from build123d import *

# Parameters (mm, degrees)
PLATE_OUTLINE_SKETCH_R = 10
BASE_PLATE_DEPTH       = 30
POCKET_SKETCH_R        = 10
POCKET_DEPTH           = 5


with BuildPart() as part:
    # Plate Outline Sketch → Base Plate (new body)
    with BuildSketch(Plane(origin=(0, 0, 0), x_dir=(1, 0, 0), z_dir=(0, 1, 0))):
        with BuildLine():
            ThreePointArc((-90, -88), (-80.846522891, -104.803361008), (-61.764705882, -106.225803982))
            ThreePointArc((-61.764705882, -106.225803982), (0, -92.919333848), (61.764705882, -106.225803982))
            ThreePointArc((61.764705882, -106.225803982), (80.846522891, -104.803361008), (90, -88))
            Line((90, -88), (90, -31.013960492))
            ThreePointArc((90, -31.013960492), (86.763523469, -20.105968885), (78.101571911, -12.728323162))
            Line((78.101571911, -12.728323162), (8.101571911, 18.28563733))
            ThreePointArc((8.101571911, 18.28563733), (0, 20), (-8.101571911, 18.28563733))
            Line((-8.101571911, 18.28563733), (-78.101571911, -12.728323162))
            ThreePointArc((-78.101571911, -12.728323162), (-86.763523469, -20.105968885), (-90, -31.013960492))
            Line((-90, -31.013960492), (-90, -88))
        make_face()
        with Locations(Location((70, -88, 0), (0, 0, 270))):
            Circle(PLATE_OUTLINE_SKETCH_R, mode=Mode.SUBTRACT)
        with Locations(Location((-70, -88, 0), (0, 0, 270))):
            Circle(PLATE_OUTLINE_SKETCH_R, mode=Mode.SUBTRACT)
        with Locations(Location((0, 0, 0), (0, 0, 270))):
            Circle(PLATE_OUTLINE_SKETCH_R, mode=Mode.SUBTRACT)
        with BuildLine():
            ThreePointArc((55.144271878, -90.075413685), (61.617206501, -75.560997904), (77.5, -75.009618943))
            ThreePointArc((77.5, -75.009618943), (82.5, -75.009618943), (85, -70.679491924))
            Line((85, -70.679491924), (85, -35.770992672))
            ThreePointArc((85, -35.770992672), (81.864151045, -25.019229582), (73.439959048, -17.639056998))
            Line((73.439959048, -17.639056998), (22.032686199, 6.289732813))
            ThreePointArc((22.032686199, 6.289732813), (17.05201209, 5.850545589), (14.942022328, 1.317561671))
            ThreePointArc((14.942022328, 1.317561671), (0, -15), (-14.942022328, 1.317561671))
            ThreePointArc((-14.942022328, 1.317561671), (-17.05201209, 5.850545589), (-22.032686199, 6.289732813))
            Line((-22.032686199, 6.289732813), (-73.439959048, -17.639056998))
            ThreePointArc((-73.439959048, -17.639056998), (-81.864151045, -25.019229582), (-85, -35.770992672))
            Line((-85, -35.770992672), (-85, -70.679491924))
            ThreePointArc((-85, -70.679491924), (-82.5, -75.009618943), (-77.5, -75.009618943))
            ThreePointArc((-77.5, -75.009618943), (-61.617206501, -75.560997904), (-55.144271878, -90.075413685))
            ThreePointArc((-55.144271878, -90.075413685), (-53.374733144, -94.623708504), (-48.573254036, -95.497808883))
            ThreePointArc((-48.573254036, -95.497808883), (0, -87.415527975), (48.573254036, -95.497808883))
            ThreePointArc((48.573254036, -95.497808883), (53.374733144, -94.623708504), (55.144271878, -90.075413685))
        make_face(mode=Mode.SUBTRACT)
    extrude(amount=BASE_PLATE_DEPTH)

    # Pocket Sketch → Pocket (add)
    with BuildSketch(Plane.XZ):
        with BuildLine():
            Line((-90, 88), (-90, 31.013960492))
            ThreePointArc((-90, 31.013960492), (-86.763523469, 20.105968885), (-78.101571911, 12.728323162))
            Line((-78.101571911, 12.728323162), (-8.101571911, -18.28563733))
            ThreePointArc((-8.101571911, -18.28563733), (0, -20), (8.101571911, -18.28563733))
            Line((8.101571911, -18.28563733), (78.101571911, 12.728323162))
            ThreePointArc((78.101571911, 12.728323162), (86.763523469, 20.105968885), (90, 31.013960492))
            Line((90, 31.013960492), (90, 88))
            ThreePointArc((90, 88), (80.846522891, 104.803361008), (61.764705882, 106.225803982))
            ThreePointArc((61.764705882, 106.225803982), (0, 92.919333848), (-61.764705882, 106.225803982))
            ThreePointArc((-61.764705882, 106.225803982), (-80.846522891, 104.803361008), (-90, 88))
        make_face()
        with Locations(Location((-70, 88, 0), (0, 0, 90))):
            Circle(POCKET_SKETCH_R, mode=Mode.SUBTRACT)
        with Locations(Location((0, 0, 0), (0, 0, 90))):
            Circle(POCKET_SKETCH_R, mode=Mode.SUBTRACT)
        with Locations(Location((70, 88, 0), (0, 0, 90))):
            Circle(POCKET_SKETCH_R, mode=Mode.SUBTRACT)
    extrude(amount=-POCKET_DEPTH)


solid = part.part
CAD build for the part. Positions are in the model's coordinates, mm. A direction names the side the tool comes from. Give positions to 0.01 mm unless a question says otherwise; leave off trailing zeros. Loops run counter-clockwise (first coordinate to the right, second up) from the corner with the lowest first, then second, coordinate; pieces in that order, holes last. Notation, with made-up numbers: M 28,7.25 L 61,7.25 A18 cw 61,18.25 Z; hole C -14,-28 d1. An arc over 180 degrees is marked long. Write each question's results on one line, items separated by ' | '.
Q1. Band-saw the part on C-C on x = 51.5. Write the cut outline in (y, z).
Geometry check:
outline: M 0,0.94 L 30,0.94 L 30,7.43 L 5,7.43 L 5,95.59 L 30,95.59 L 30,102.04 L 0,102.04 Z
Q2. Band-saw the part on B-B on y = 22. Give the number of separate pieces and of enclosed holes in the cut face, and give its area (3 significant figures).
Geometry check:
separate pieces: 1 | enclosed holes: 4 | area: 4,160 mm²
Q3. Mould opens along X. For faces 3 (the face through (0, 15, -20)), 4 (the face through (-86.675, 14.79, 19.971)), 5 (the face through (86.85, 14.79, 20.24)), 6 (the face through (53.32, 17.32, 94.67)) say: pulls with the +X half, pulls with the -X half, needs draft (parallel to the pull), parting line crosses it, or undercut.
Geometry check:
face 3: parting line crosses it | face 4: pulls with the -X half | face 5: pulls with the +X half | face 6: undercut
Q4. Flat gauge pins, fed straight in: P1, Ø1, axis at x = -41, y = 5, coming from the -Z side; P2, Ø8, axis at x = -67, z = 61, coming from the -Y side; P3, Ø1.5, axis at x = 54.5, y = 20, coming from the -Z side; P4, Ø2, axis at x = 12, z = 35.5, coming from the +Y side. Where does each tip first touch, or does it go through?
Geometry check:
P1: stops at z = -3.93 | P2: stops at y = 0 | P3: stops at z = 1.94 | P4: stops at y = 5
Q5. Which spindle directions (+Z, -Z, +X, -X, +Y, -Y) get a long thin tool onto all of the face, cutting with end or side? Do faces 1 (the face through (-81.78, 17.32, 24.89)), 2 (the face through (-0.89, 14.79, 92.92)). Say none if no direction does.
Geometry check:
face 1: +Y | face 2: +Z, +Y, -Y
Q6. Band-saw the part on A-A on x = 0. Write the cut outline in (y, z).
Geometry check:
outline: M 0,-20 L 30,-20 L 30,-10 L 0,-10 Z; M 0,10 L 30,10 L 30,15 L 5,15 L 5,87.42 L 30,87.42 L 30,92.92 L 0,92.92 Z
Q7. Band-saw the part on D-D on x = -70. Write the cut outline in (y, z), and give its area (3 significant figures).
Geometry check:
outline: M 0,9.14 L 30,9.14 L 30,16.04 L 5,16.04 L 5,73 L 30,73 L 30,78 L 0,78 Z; M 0,98 L 30,98 L 30,108 L 0,108 Z | area: 942 mm²
Q8. Probe probe 1 along X at (y, z) = (28, 57); probe 2 along X at (y, z) = (18.25, 0); probe 3 along Z at (x, y) = (63.5, 20). List the from-to ranges inside material, lowest first.
Geometry check:
probe 1: x = -90 to -85, 85 to 90 | probe 2: x = -49.37 to -35.55, -15 to -10, 10 to 15, 35.55 to 49.37 | probe 3: z = 6.26 to 13.01, 74.48 to 80.4, 95.6 to 106.91
